from build123d import *

# Parameters (mm, degrees)
BOSS_EXTRUDE1_DEPTH = 12


with BuildPart() as part:
    # Sketch1 → Boss-Extrude1 (new body)
    with BuildSketch(Plane.XY):
        with BuildLine():
            Line((0, 0), (40, 0))
            Line((40, 0), (40, 30))
            ThreePointArc((40, 30), (37.071067812, 37.071067812), (30, 40))
            Line((30, 40), (10, 40))
            ThreePointArc((10, 40), (2.928932188, 37.071067812), (0, 30))
            Line((0, 30), (0, 0))
        make_face()
    extrude(amount=BOSS_EXTRUDE1_DEPTH)


solid = part.part
Check sheet for the modelled part. Datum: model origin and axes. Units: mm. Coordinates: 2 decimals unless noted, no trailing zeros. Loops run counter-clockwise (first coordinate to the right, second up) from the corner with the lowest first, then second, coordinate; pieces in that order, holes last. Notation, with made-up numbers: (53.25, 52.25) -> (78.25, 52.25) arc R20 cw to (78.25, 91.25) -> close; hole circle Ø9 at (-35, 9). An arc over 180 degrees is marked (long way). Answer in a Markdown table with one row per item.
1. Sectioned sample at B-B, the plane x = 4. Record the boundary of the cut face in (y, z), then the cut area to 3 significant figures.
Check values:
| item | result |
|---|---|
| outline | (0, 0) -> (38, 0) -> (38, 12) -> (0, 12) -> close |
| area | 456 mm2 |
2. Material ranges on line 1 along X through (y, z) = (35, 8.5); line 2 along Y through (x, z) = (7, 10.5); line 3 along Y through (x, z) = (32.5, 8), recorded low to high. Write a range as [from, to].
Check values:
| item | result |
|---|---|
| line 1 | x = [1.34, 38.66] |
| line 2 | y = [0, 39.54] |
| line 3 | y = [0, 39.68] |
3. Sectioned sample at A-A, the plane z = 9. Record the boundary of the cut face in (x, y), then the cut area to 3 significant figures.
Check values:
| item | result |
|---|---|
| outline | (0, 0) -> (40, 0) -> (40, 30) arc R10 ccw to (30, 40) -> (10, 40) arc R10 ccw to (0, 30) -> close |
| area | 1,560 mm2 |
4. Sectioned sample at C-C, the plane y = 34.5. Record the boundary of the cut face in (x, z).
Check values:
| item | result |
|---|---|
| outline | (1.07, 0) -> (38.93, 0) -> (38.93, 12) -> (1.07, 12) -> close |
